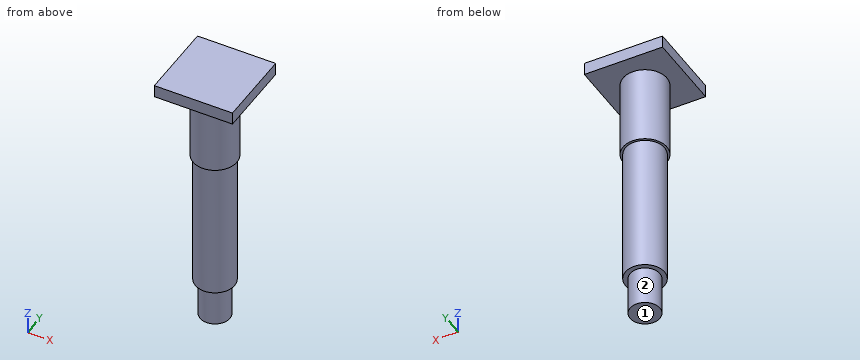
from build123d import *

# Parameters (mm, degrees)
SKETCH_1_R      = 12.5
EXTRUDE_1_DEPTH = 90
SKETCH_2_R      = 14
EXTRUDE_2_DEPTH = 50
SKETCH_3_W      = 50
SKETCH_3_H      = 50
EXTRUDE_3_DEPTH = 8
SKETCH_4_R      = 9.5
EXTRUDE_4_DEPTH = 25


with BuildPart() as part:
    # 草图1 → 凸台-拉伸1 (new body)
    with BuildSketch(Plane.XY):
        with Locations(Location((0, 0, 0), (0, 0, 180))):
            Circle(SKETCH_1_R)
    extrude(amount=EXTRUDE_1_DEPTH)

    # 草图2 → 凸台-拉伸2 (add)
    with BuildSketch(Plane.XY.offset(90)):
        Circle(SKETCH_2_R)
    extrude(amount=EXTRUDE_2_DEPTH)

    # 草图3 → 凸台-拉伸3 (add)
    with BuildSketch(Plane.XY.offset(140)):
        Rectangle(SKETCH_3_W, SKETCH_3_H)
    extrude(amount=EXTRUDE_3_DEPTH)

    # 草图4 → 凸台-拉伸4 (add)
    with BuildSketch(Plane(origin=(0, 0, 0), x_dir=(-1, 0, 0), z_dir=(0, 0, -1))):
        Circle(SKETCH_4_R)
    extrude(amount=EXTRUDE_4_DEPTH)


solid = part.part
Geometry: final body of the model. Coordinates: model frame, mm. Face numbers are marked on the shaded views. A direction names the side the tool comes from. Round coordinates to 2 decimals unless told otherwise and drop trailing zeros. Write each loop counter-clockwise with the first axis right and the second up, starting at its lowest first coordinate (ties: lowest second). Pieces come first, ordered by that corner, then holes. Notation, with made-up numbers: M -10.75,-35.5 L 0.25,-35.5 A10 ccw 0.25,-23.5 Z; hole C 40,-7.75 d7. An arc over 180 degrees is marked long. Write item = value, one per line.
Item 1: Section query C-C on z = 125. Return loops of the section in (x, y), then the cut area to 3 significant figures.
Findings:
outline = C 0,0 d28
area = 616 mm^2
Item 2: Material intervals for line 1 along Z through (x, y) = (-17, 11.5); line 2 along Z through (x, y) = (1.5, 12.5); line 3 along X through (y, z) = (-8, 62.5), sorted ascending. Write a range as [from, to].
Findings:
line_1 = [140, 148]
line_2 = [90, 148]
line_3 = [-9.6, 9.6]
Item 3: Pin query (flat end, axial travel): P1, Ø6, axis at x = -6, y = -9, coming from the -Z side; P2, Ø10, axis at x = -14, z = 31.5, coming from the +Y side; P3, Ø1.5, axis at x = 7.5, z = 95, coming from the -Y side; P4, Ø12, axis at y = 5, z = 48.5, coming from the +X side. Return the tip coordinate at first contact, or that it passes through.
Findings:
P1 = -25
P2 = 8.67
P3 = -12.27
P4 = 12.5
Item 4: Section query D-D on z = 25. Return loops of the section in (x, y).
Findings:
outline = C 0,0 d25
Item 5: Access query for the marked faces 1 and 2. Directions: +Z, -Z, +X, -X, +Y, -Y. A direction counts if a zero-diameter tool reaches every point of the face in a straight line with its end or side. Return the directions, or none.
Findings:
face_1 = -Z, +X, -X, +Y, -Y
face_2 = -Z
Item 6: Section query A-A on x = 0. Return loops of the section in (y, z), then the cut area to 4 significant figures.
Findings:
outline = M -25,140 L -14,140 L -14,90 L -12.5,90 L -12.5,0 L -9.5,0 L -9.5,-25 L 9.5,-25 L 9.5,0 L 12.5,0 L 12.5,90 L 14,90 L 14,140 L 25,140 L 25,148 L -25,148 Z
area = 4,525 mm^2
